Input: dimensioned drawing with shaded views. Units: mm. Origin: part minimum x, y, z. A direction names the side the tool comes from. Round coordinates to 2 decimals unless told otherwise and drop trailing zeros. Write each loop counter-clockwise with the first axis right and the second up, starting at its lowest first coordinate (ties: lowest second). Pieces come first, ordered by that corner, then holes. Notation, with made-up numbers: M 46.25,37 L 56.25,37 A28 cw 56.25,60 Z; hole C 79,68.5 d5. An arc over 180 degrees is marked long. Answer in a Markdown table with one row per item. Add a question column.
Item 1: Cut plane D-D on y = 18. Return loops of the section in (x, z), and give its area (3 significant figures).
Item 2: Material intervals for probe 1 along Y at (x, z) = (21, 26.6); probe 2 along Z at (x, y) = (36.5, 27); probe 3 along Z at (x, y) = (7, 22.5), sorted ascending.
Item 3: Cut plane C-C on x = 5. Return loops of the section in (y, z), and give its area (3 significant figures).
Item 4: Mould query, pull axis X, two halves, no side actions, for the marked faces 4, 5 and 6. Classes: released by +X, released by -X, zero draft, split by the parting line, or undercut.
Item 5: Contact query for flat-ended pins moving along their axis: pin 1 (10.5 mm diameter, centred on x = 5, y = 21, fed in from +Z); pin 2 (7 mm diameter, centred on x = 21, y = 5, fed in from +Z); pin 3 (2 mm diameter, centred on y = 21, z = 17.5, fed in from -X); pin 4 (10 mm diameter, centred on y = 8, z = 3.5, fed in from -X). Output: stop coordinate, or through.
Item 6: Cut plane A-A on x = 21. Return loops of the section in (y, z).
Item 7: Set-up query: the marked faces 1, 2 and 3. Return all of +Z, -Z, +X, -X, +Y, -Y with unobstructed straight access to the full face (end or side cutting, diameter ignored); none if empty.
Item 8: Cut plane B-B on y = 6.5. Return loops of the section in (x, z), and give its area (3 significant figures).
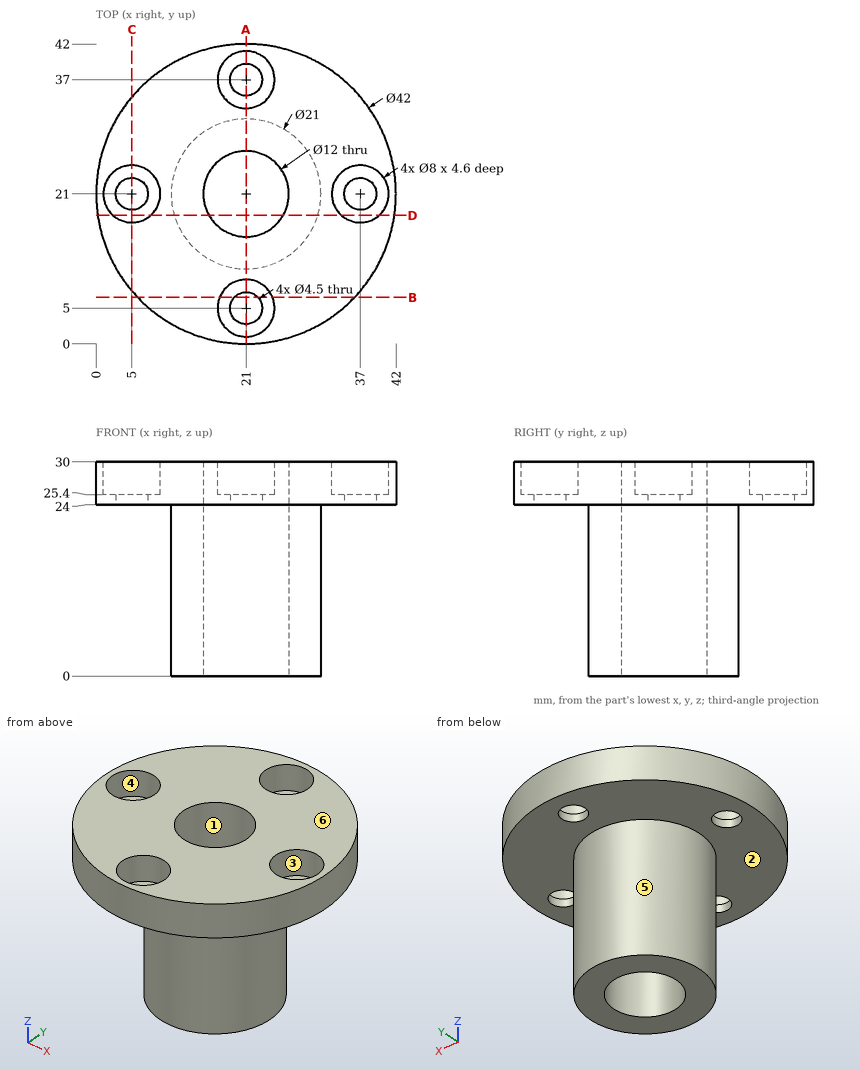
Results below:
| question | item | result |
|---|---|---|
| 1 | outline | M 0.22,24 L 10.94,24 L 10.94,0 L 15.8,0 L 15.8,30 L 7.65,30 L 7.65,25.4 L 2.35,25.4 L 2.35,30 L 0.22,30 Z; M 26.2,0 L 31.06,0 L 31.06,24 L 41.78,24 L 41.78,30 L 39.65,30 L 39.65,25.4 L 34.35,25.4 L 34.35,30 L 26.2,30 Z |
| 1 | area | 372 mm2 |
| 2 | probe 1 | 0 to 1, 9 to 15, 27 to 33, 41 to 42 |
| 2 | probe 2 | 24 to 30 |
| 2 | probe 3 | 24 to 25.4 |
| 3 | outline | M 7.4,24 L 18.75,24 L 18.75,25.4 L 17,25.4 L 17,30 L 7.4,30 Z; M 23.25,24 L 34.6,24 L 34.6,30 L 25,30 L 25,25.4 L 23.25,25.4 Z |
| 3 | area | 120 mm2 |
| 4 | face 4 | undercut |
| 4 | face 5 | split by the parting line |
| 4 | face 6 | zero draft |
| 5 | pin 1 | z = 30 |
| 5 | pin 2 | z = 25.4 |
| 5 | pin 3 | x = 10.5 |
| 5 | pin 4 | x = 14.2 |
| 6 | outline | M 0,24 L 2.75,24 L 2.75,25.4 L 1,25.4 L 1,30 L 0,30 Z; M 7.25,24 L 10.5,24 L 10.5,0 L 15,0 L 15,30 L 9,30 L 9,25.4 L 7.25,25.4 Z; M 27,0 L 31.5,0 L 31.5,24 L 34.75,24 L 34.75,25.4 L 33,25.4 L 33,30 L 27,30 Z; M 39.25,24 L 42,24 L 42,30 L 41,30 L 41,25.4 L 39.25,25.4 Z |
| 7 | face 1 | +Z, -Z |
| 7 | face 2 | -Z |
| 7 | face 3 | +Z |
| 8 | outline | M 5.81,24 L 19.32,24 L 19.32,25.4 L 17.29,25.4 L 17.29,30 L 5.81,30 Z; M 22.68,24 L 36.19,24 L 36.19,30 L 24.71,30 L 24.71,25.4 L 22.68,25.4 Z |
| 8 | area | 143 mm2 |
